Part model, mm, in its own coordinate system. A direction names the side the tool comes from. Give positions to 0.01 mm unless a question says otherwise; leave off trailing zeros. Write each loop counter-clockwise with the first axis right and the second up, starting at its lowest first coordinate (ties: lowest second). Pieces come first, ordered by that corner, then holes.
```python
from build123d import *

# Parameters (mm, degrees)
SKETCH_1_W          = 27
SKETCH_1_H          = 16
EXTRUDE_1_DEPTH     = 4
SKETCH_2_R          = 0.75
SKETCH_2_R_2        = 1.59
CUT_EXTRUDE_2_DEPTH = 4
CUT_EXTRUDE_3_DEPTH = 4
CUT_EXTRUDE_4_DEPTH = 2


with BuildPart() as part:
    # 草图1 → 凸台-拉伸1 (new body)
    with BuildSketch(Plane.XY):
        with Locations((3.898916968, -3.881768953)):
            Rectangle(SKETCH_1_W, SKETCH_1_H)
    extrude(amount=EXTRUDE_1_DEPTH)

    # 草图2 → 切除-拉伸2 (cut)
    with BuildSketch(Plane.XY.offset(4)):
        with Locations((1.199905932, -1.781578746)):
            Circle(SKETCH_2_R)
        with Locations((1.122511443, -6.056778774)):
            Circle(SKETCH_2_R)
        with Locations((9.465404763, -4.069510677)):
            Circle(SKETCH_2_R_2)
    extrude(amount=-CUT_EXTRUDE_2_DEPTH, mode=Mode.SUBTRACT)

    # 草图3 → 切除-拉伸3 (cut)
    with BuildSketch(Plane.XY.offset(4)):
        with BuildLine():
            Line((6.931862452, -2.481455291), (9.464184068, -2.479511145))
            ThreePointArc((9.464184068, -2.479511145), (7.875405231, -4.070731371), (9.466625457, -5.659510208))
            Line((9.466625457, -5.659510208), (6.934303841, -5.661454354))
            ThreePointArc((6.934303841, -5.661454354), (5.343083615, -4.072675517), (6.931862452, -2.481455291))
        make_face()
        with BuildLine():
            Line((-1.276445305, -7.332757851), (0.601227077, -5.517554692))
            ThreePointArc((0.601227077, -5.517554692), (0.583287361, -6.578063139), (1.643795809, -6.596002856))
            Line((1.643795809, -6.596002856), (-0.233876574, -8.411206015))
            ThreePointArc((-0.233876574, -8.411206015), (-1.294385021, -8.393266299), (-1.276445305, -7.332757851))
        make_face()
        with BuildLine():
            Line((-1.145979965, -0.556904877), (0.678621567, -2.320802827))
            ThreePointArc((0.678621567, -2.320802827), (0.660681851, -1.26029438), (1.721190298, -1.242354664))
            Line((1.721190298, -1.242354664), (-0.103411234, 0.521543286))
            ThreePointArc((-0.103411234, 0.521543286), (-1.163919681, 0.50360357), (-1.145979965, -0.556904877))
        make_face()
    extrude(amount=-CUT_EXTRUDE_3_DEPTH, mode=Mode.SUBTRACT)

    # 草图5 → 切除-拉伸4 (cut)
    with BuildSketch(Plane(origin=(0, 0, 0), x_dir=(-1, 0, 0), z_dir=(0, 0, -1))):
        with BuildLine():
            Line((-9.463485432, -1.569511413), (-6.931163815, -1.57145556))
            ThreePointArc((-6.931163815, -1.57145556), (-4.433083883, -4.073374154), (-6.935002478, -6.571454086))
            Line((-6.935002478, -6.571454086), (-9.467324094, -6.56950994))
            ThreePointArc((-9.467324094, -6.56950994), (-11.965404026, -4.067591345), (-9.463485432, -1.569511413))
        make_face()
        with BuildLine():
            Line((-0.244111676, 0.881026007), (-2.068713208, -0.882871943))
            ThreePointArc((-2.068713208, -0.882871943), (-2.098612735, -2.650386022), (-0.331098657, -2.680285548))
            Line((-0.331098657, -2.680285548), (1.493502876, -0.916387599))
            ThreePointArc((1.493502876, -0.916387599), (1.523402402, 0.85112648), (-0.244111676, 0.881026007))
        make_face()
        with BuildLine():
            Line((-0.253704167, -5.158071971), (1.623968215, -6.97327513))
            ThreePointArc((1.623968215, -6.97327513), (1.653867742, -8.740789209), (-0.113646337, -8.770688736))
            Line((-0.113646337, -8.770688736), (-1.991318719, -6.955485577))
            ThreePointArc((-1.991318719, -6.955485577), (-2.021218246, -5.187971498), (-0.253704167, -5.158071971))
        make_face()
    extrude(amount=-CUT_EXTRUDE_4_DEPTH, mode=Mode.SUBTRACT)


solid = part.part
```
1) Saw through at A-A, the plane z = 1.6. Count the separate pieces of the cut face and the enclosed holes in it, then the cut area to 3 significant figures.
Answers follow:
separate pieces: 1
enclosed holes: 3
area: 377 mm2
2) Wall check: L1, parallel to Y at x = 9.5, z = 2.1; L2, parallel to X at y = -7.25, z = 2.25; L3, parallel to X at y = -4, z = 1.85. Give the ranges that are in metal, low to high.
Answers follow:
L1: y = -11.88 to -5.66, -2.48 to 4.12
L2: x = -9.6 to -1.19, 0.97 to 17.4
L3: x = -9.6 to 4.43, 11.96 to 17.4
3) Two-plate mould, pull along X, no slides. Class faces 3 (the face through (4, -4, 4)), 4 (the face through (-9.601, -4, 2)), 5 (the face through (8, -6, 2)): +X half, -X half, draft (parallel to the pull), parting line (faces both ways), or undercut.
Answers follow:
face 3: draft
face 4: -X half
face 5: undercut
4) 3-axis set-ups, long thin cutter, end or side, ignore diameter. For faces 1 (the face through (0.82, -0.37, 3.01)), 2 (the face through (4.434, -4.018, 0.986)): which of +Z, -Z, +X, -X, +Y, -Y reach the whole face in a straight line?
Answers follow:
face 1: +Z, -Z
face 2: -Z
5) Saw through at B-B, the plane x = 10.25. Write the cut outline in (y, z), then the cut area to 3 significant figures.
Answers follow:
outline: (-11.88, 0) - (-6.44, 0) - (-6.44, 2) - (-5.45, 2) - (-5.45, 4) - (-11.88, 4) - close; (-2.69, 2) - (-1.7, 2) - (-1.7, 0) - (4.12, 0) - (4.12, 4) - (-2.69, 4) - close
area: 49.0 mm2
